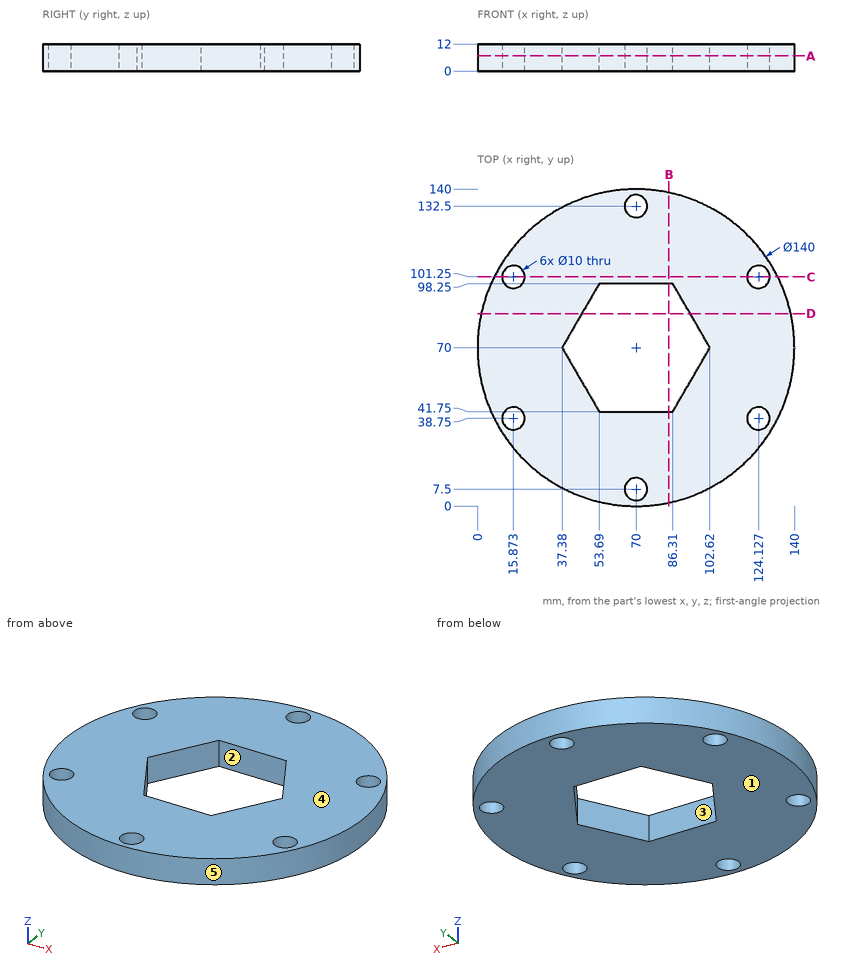
Answer from the drawing. Dimensions are ordinates in mm from the lowest x, y and z of the part. A direction names the side the tool comes from. Give positions to 0.01 mm unless a question says otherwise; leave off trailing zeros. Order: outer loops, then holes, each group sorted by start corner. A loop starts at its lowest first (then second) coordinate and runs counter-clockwise, first axis right, second up. Notation, with made-up numbers: (-6, -28.5) - (37, -28.5) arc R15 cw to (37, -1.5) - close; hole circle Ø4 at (57, 41). An arc over 180 degrees is marked (long way). One line per item, written item: value. Start each with the question number.
1) A cutting plane is placed at C-C on y = 101.25. Give the vertices of the cut face in (x, z).
2) Find the intervals of material crossed by L1, parallel to Y at x = 70, z = 6.75; L2, parallel to X at y = 97, z = 7.5 (1 decimal); L3, parallel to X at y = 94, z = 0.75 (1 decimal), in increasing order.
3) The mould has two halves that part along X. Classify the marked faces 3, 4 and 5: released by +X, released by -X, zero draft, split by the parting line, or undercut.
4) A cutting plane is placed at B-B on x = 84.5. Give the vertices of the cut face in (y, z).
5) Given pin 1 Ø1 at (y, z) = (108, 9) entering from +X; pin 2 Ø1.5 at (x, z) = (21, 6.5) entering from -Y (1 decimal); pin 3 Ø1 at (y, z) = (125.5, 4.5) entering from -X, each flat-ended and moving along its own axis, determine where each tip first touches the part or whether it passes through.
6) A tool of negligible diameter and unlimited length cuts with its end or side. For the marked faces 1 and 2, from which of +Z, -Z, +X, -X, +Y, -Y can it reach the whole face along a straight path? Write none if from no direction.
7) A cutting plane is placed at A-A on z = 6.75. Give the vertices of the cut face in (x, y).
8) A cutting plane is placed at D-D on y = 85. Give the vertices of the cut face in (x, z).
Answer sheet:
1. outline: (7.36, 0) - (10.87, 0) - (10.87, 12) - (7.36, 12) - close; (20.87, 0) - (119.13, 0) - (119.13, 12) - (20.87, 12) - close; (129.13, 0) - (132.64, 0) - (132.64, 12) - (129.13, 12) - close
2. L1: y = 0 to 2.5, 12.5 to 41.75, 98.25 to 127.5, 137.5 to 140
2. L2: x = 5.4 to 13.2, 18.5 to 53, 87 to 121.5, 126.8 to 134.6
2. L3: x = 4.2 to 51.2, 88.8 to 135.8
3. face 3: undercut
3. face 4: zero draft
3. face 5: split by the parting line
4. outline: (1.52, 0) - (41.75, 0) - (41.75, 12) - (1.52, 12) - close; (98.25, 0) - (138.48, 0) - (138.48, 12) - (98.25, 12) - close
5. pin 1: stops at x = 129.11
5. pin 2: stops at y = 19.3
5. pin 3: stops at x = 26.7
6. face 1: -Z, +X, -X, +Y, -Y
6. face 2: +Z, -Z
7. outline: circle Ø140 at (70, 70); hole circle Ø10 at (15.87, 38.75); hole circle Ø10 at (15.87, 101.25); hole (37.38, 70) - (53.69, 41.75) - (86.31, 41.75) - (102.62, 70) - (86.31, 98.25) - (53.69, 98.25) - close; hole circle Ø10 at (70, 7.5); hole circle Ø10 at (70, 132.5); hole circle Ø10 at (124.13, 38.75); hole circle Ø10 at (124.13, 101.25)
8. outline: (1.63, 0) - (46.04, 0) - (46.04, 12) - (1.63, 12) - close; (93.96, 0) - (138.37, 0) - (138.37, 12) - (93.96, 12) - close
